For this review, take the finished solid that the model builds, in its own axes (mm). A direction names the side the tool comes from. Coordinates: 2 decimals unless noted, no trailing zeros. Loops run counter-clockwise (first coordinate to the right, second up) from the corner with the lowest first, then second, coordinate; pieces in that order, holes last. Notation, with made-up numbers: (16.5, 36.5) - (39.5, 36.5) arc R35 cw to (39.5, 70.5) - close; hole circle Ø4 at (64.5, 75.25). An arc over 180 degrees is marked (long way). Use one line per item in the form item = value. Start each with the question number.
1. Add section A-A on x = 0. Give the boundary of the cut face in (y, z), and give its area (4 significant figures).
2. To check wall thickness, follow probe 1 along Z at (x, y) = (-1.75, -5.5); probe 2 along X at (y, z) = (-0.25, 17); probe 3 along Y at (x, z) = (-3.75, 28.5). State the ranges of each line that lie inside material, in increasing order.
3. For pin 1 Ø4 at (y, z) = (0.5, 6) entering from +X; pin 2 Ø5 at (x, y) = (-0.5, -1) entering from -Z; pin 3 Ø3 at (y, z) = (5, 36.5) entering from +X; pin 4 Ø2 at (x, z) = (-1.5, 27.5) entering from -Y, all flat-tipped, find the tip position at first contact; note any pin that passes through.
4. Add section C-C on z = 32. Give the boundary of the cut face in (x, y), and give its area (3 significant figures).
5. Machinability: for faces 1 (the face through (-2, 5, 46)), 2 (the face through (0, 0, 0)), 3 (the face through (0.867, -3.905, 2.986)), which of the approach directions +Z, -Z, +X, -X, +Y, -Y give a long, thin tool a straight path to every point of the face, cutting with its end or side? Answer none if there is none.
```python
from build123d import *

# Parameters (mm, degrees)
SKETCH1_R               = 5
BOSS_EXTRUDE1_DEPTH     = 46
SKETCH2_R               = 7
BOSS_EXTRUDE2_DEPTH     = 2
CHAMFER1_SIZE           = 0.5
SKETCH3_R               = 14
SKETCH3_R_2             = 4
CUT_EXTRUDE_THIN1_DEPTH = 2


with BuildPart() as part:
    # Sketch1 → Boss-Extrude1 (new body)
    with BuildSketch(Plane.XY):
        Circle(SKETCH1_R)
    extrude(amount=BOSS_EXTRUDE1_DEPTH)

    # Sketch2 → Boss-Extrude2 (add)
    with BuildSketch(Plane.XY.offset(46)):
        Circle(SKETCH2_R)
    extrude(amount=BOSS_EXTRUDE2_DEPTH)

    # Chamfer1
    chamfer1_edges = [part.edges().sort_by_distance(p)[0] for p in [
        (-5, 0, 0),
        (-7, 0, 48),
    ]]
    chamfer(chamfer1_edges, length=CHAMFER1_SIZE)

    # Sketch3 → Cut-Extrude-Thin1 (cut)
    with BuildSketch(Plane(origin=(0, 0, 2), x_dir=(-1, 0, 0), z_dir=(0, 0, -1))):
        Circle(SKETCH3_R)
        Circle(SKETCH3_R_2, mode=Mode.SUBTRACT)
    extrude(amount=-CUT_EXTRUDE_THIN1_DEPTH, mode=Mode.SUBTRACT)


solid = part.part
```
Conclusion:
q1.outline = (-7, 46) - (-5, 46) - (-5, 4) - (-4, 4) - (-4, 2) - (-5, 2) - (-5, 0.5) - (-4.5, 0) - (4.5, 0) - (5, 0.5) - (5, 2) - (4, 2) - (4, 4) - (5, 4) - (5, 46) - (7, 46) - (7, 47.5) - (6.5, 48) - (-6.5, 48) - (-7, 47.5) - close
q1.area = 483.5 mm^2
q2.probe_1 = 46 to 48
q2.probe_2 = -4.99 to 4.99
q2.probe_3 = -3.31 to 3.31
q3.pin_1 = 5
q3.pin_2 = 0
q3.pin_3 = 3.57
q3.pin_4 = -4.97
q4.outline = circle Ø10 at (0, 0)
q4.area = 78.5 mm^2
q5.face_1 = -Z
q5.face_2 = -Z, +X, -X, +Y, -Y
q5.face_3 = none
